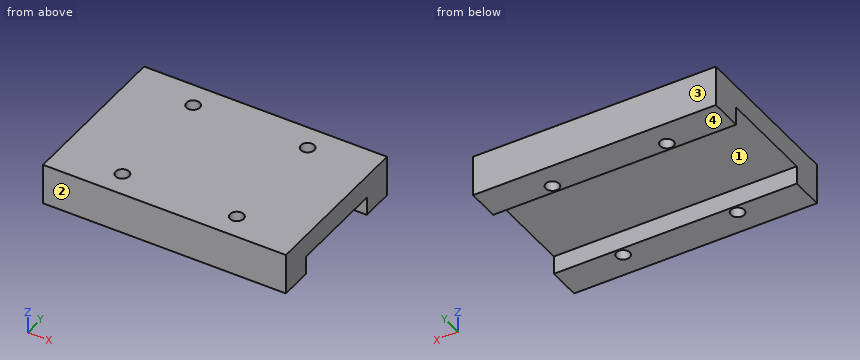
from build123d import *

# Parameters (mm, degrees)
SKETCH1_W             = 59.4
SKETCH1_H             = 40
BOSS_EXTRUDE1_DEPTH   = 10
SKETCH2_W             = 9
SKETCH2_H             = 24
CUT_EXTRUDE1_DEPTH    = 64.469362688
M4_TAPPED_HOLE1_D     = 3.3
M4_TAPPED_HOLE1_DEPTH = 10.1
M4_TAPPED_HOLE1_TIP   = 0.991420021


with BuildPart() as part:
    # Sketch1 → Boss-Extrude1 (new body)
    with BuildSketch(Plane.XY):
        Rectangle(SKETCH1_W, SKETCH1_H)
    extrude(amount=BOSS_EXTRUDE1_DEPTH)

    # Sketch2 → Cut-Extrude1 (cut, through all)
    with BuildSketch(Plane.ZY.offset(29.7)):
        Rectangle(SKETCH2_W, SKETCH2_H)
    extrude(amount=-CUT_EXTRUDE1_DEPTH, mode=Mode.SUBTRACT)

    # M4 Tapped Hole1
    with Locations(Plane.XY.offset(10)):
        with Locations((-14, 14), (14, 14), (14, -14), (-14, -14)):
            Hole(M4_TAPPED_HOLE1_D / 2, depth=M4_TAPPED_HOLE1_DEPTH)
            with Locations((0, 0, -(M4_TAPPED_HOLE1_DEPTH + M4_TAPPED_HOLE1_TIP / 2))):  # 118° drill point
                Cone(0, M4_TAPPED_HOLE1_D / 2, M4_TAPPED_HOLE1_TIP, mode=Mode.SUBTRACT)


solid = part.part
Model file for the job. Use its own axes, mm. Face numbers are marked on the shaded views. Give positions to 0.01 mm unless a question says otherwise; leave off trailing zeros. Loops run counter-clockwise (first coordinate to the right, second up) from the corner with the lowest first, then second, coordinate; pieces in that order, holes last.
1) Saw through at B-B (y = -14). Write the cut outline in (x, z).
2) Wall check: line 1 (Y direction, x = -14, z = 7); line 2 (Y direction, x = 14, z = 3.5); line 3 (Y direction, x = 10, z = 1). Give the ranges that are in metal, low to high.
3) Flat gauge pin, fed straight in: pin 1 Ø10 at (x, y) = (-1.5, -2) entering from -Z. Where does the tip first touch, or does it go through?
4) Pull direction Y, two halves, no side cores. Call the marked faces 1, 2, 3 and 4: +Y half, -Y half, draft (parallel to the pull), parting line (faces both ways), or undercut.
5) Saw through at A-A (z = 1.75). Write the cut outline in (x, y), plus the area to 3 significant figures.
6) Saw through at D-D (x = 21). Write the cut outline in (y, z), plus the area to 3 significant figures.
7) Saw through at C-C (x = 14). Write the cut outline in (y, z).
Answer block:
1. outline: (-29.7, 0) - (-15.65, 0) - (-15.65, 10) - (-29.7, 10) - close; (-12.35, 0) - (12.35, 0) - (12.35, 10) - (-12.35, 10) - close; (15.65, 0) - (29.7, 0) - (29.7, 10) - (15.65, 10) - close
2. line 1: y = -20 to -15.65, -12.35 to 12.35, 15.65 to 20
2. line 2: y = -20 to -15.65, -12.35 to -12, 12 to 12.35, 15.65 to 20
2. line 3: y = -20 to -12, 12 to 20
3. pin 1: stops at z = 4.5
4. face 1: undercut
4. face 2: -Y half
4. face 3: +Y half
4. face 4: draft
5. outline: (-29.7, -20) - (29.7, -20) - (29.7, -12) - (-29.7, -12) - close; (-29.7, 12) - (29.7, 12) - (29.7, 20) - (-29.7, 20) - close; hole circle Ø3.3 at (-14, -14); hole circle Ø3.3 at (-14, 14); hole circle Ø3.3 at (14, -14); hole circle Ø3.3 at (14, 14)
5. area: 916 mm2
6. outline: (-20, 0) - (-12, 0) - (-12, 4.5) - (12, 4.5) - (12, 0) - (20, 0) - (20, 10) - (-20, 10) - close
6. area: 292 mm2
7. outline: (-20, 0) - (-15.65, 0) - (-15.65, 10) - (-20, 10) - close; (-12.35, 0) - (-12, 0) - (-12, 4.5) - (12, 4.5) - (12, 0) - (12.35, 0) - (12.35, 10) - (-12.35, 10) - close; (15.65, 0) - (20, 0) - (20, 10) - (15.65, 10) - close
